from build123d import *

# Parameters (mm, degrees)
SKETCH1_W           = 50
SKETCH1_H           = 45
BOSS_EXTRUDE1_DEPTH = 6
SKETCH2_R           = 4.5
CUT_EXTRUDE1_DEPTH  = 6
CHAMFER1_SIZE       = 10


with BuildPart() as part:
    # Sketch1 → Boss-Extrude1 (new body)
    with BuildSketch(Plane.XY):
        Rectangle(SKETCH1_W, SKETCH1_H)
    extrude(amount=BOSS_EXTRUDE1_DEPTH)

    # Sketch2 → Cut-Extrude1 (cut)
    with BuildSketch(Plane.XY.offset(6)):
        with Locations((0, -7.5)):
            Circle(SKETCH2_R)
    extrude(amount=-CUT_EXTRUDE1_DEPTH, mode=Mode.SUBTRACT)

    # Chamfer1
    chamfer1_edges = [part.edges().sort_by_distance(p)[0] for p in [
        (25, -22.5, 3),
        (-25, -22.5, 3),
    ]]
    chamfer(chamfer1_edges, length=CHAMFER1_SIZE)


solid = part.part
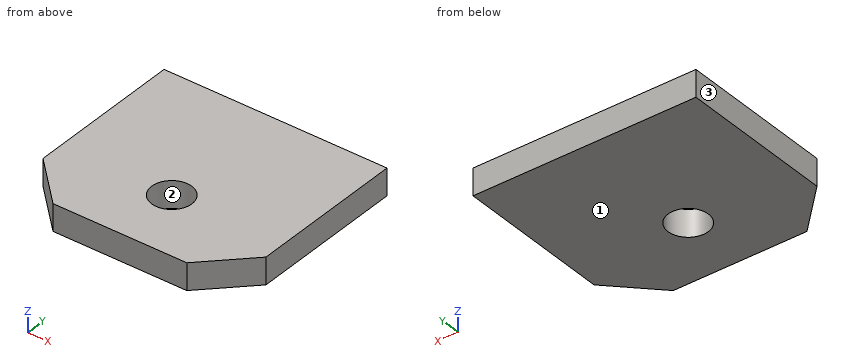
Source: CAD feature listing. Evaluate the final solid. Frame: model axes, mm. Face numbers are marked on the shaded views. Round coordinates to 2 decimals unless told otherwise and drop trailing zeros. Loops run counter-clockwise (first coordinate to the right, second up) from the corner with the lowest first, then second, coordinate; pieces in that order, holes last. Notation, with made-up numbers: (9, 41) - (33, 41) arc R25 cw to (33, 55) - close; hole circle Ø8 at (-26, -32.5). An arc over 180 degrees is marked (long way). Write item = value, one per line. Start each with the question number.
(1) Section query B-B, the plane y = -7.5. Output: boundary loops of the cut face in (x, z).
(2) Pull-direction query (X, two-part tool) for the marked faces 1, 2 and 3; classes: +X half, -X half, draft (parallel to the pull), parting line (faces both ways), or undercut.
(3) Section query A-A, the plane x = 0. Output: boundary loops of the cut face in (y, z).
(4) Ray query, line 1 along Y through (x, z) = (0, 2.8); line 2 along X through (y, z) = (-6, 3.2); line 3 along X through (y, z) = (-15, 5.65). Return the intervals inside material, ascending. Write a range as from..to.
(5) Section query C-C, the plane z = 1.1. Output: boundary loops of the cut face in (x, y).
(6) Section query D-D, the plane y = -14.5. Output: boundary loops of the cut face in (x, z), plus the area to 3 significant figures.
Conclusion:
q1.outline = (-25, 0) - (-4.5, 0) - (-4.5, 6) - (-25, 6) - close; (4.5, 0) - (25, 0) - (25, 6) - (4.5, 6) - close
q2.face_1 = draft
q2.face_2 = undercut
q2.face_3 = -X half
q3.outline = (-22.5, 0) - (-12, 0) - (-12, 6) - (-22.5, 6) - close; (-3, 0) - (22.5, 0) - (22.5, 6) - (-3, 6) - close
q4.line_1 = -22.5..-12, -3..22.5
q4.line_2 = -25..-4.24, 4.24..25
q4.line_3 = -22.5..22.5
q5.outline = (-25, -12.5) - (-15, -22.5) - (15, -22.5) - (25, -12.5) - (25, 22.5) - (-25, 22.5) - close; hole circle Ø9 at (0, -7.5)
q6.outline = (-23, 0) - (23, 0) - (23, 6) - (-23, 6) - close
q6.area = 276 mm2
